CAD build for the part. Positions are in the model's coordinates, mm. A direction names the side the tool comes from. Coordinates: 2 decimals unless noted, no trailing zeros. Order: outer loops, then holes, each group sorted by start corner. A loop starts at its lowest first (then second) coordinate and runs counter-clockwise, first axis right, second up. Notation, with made-up numbers: M -13,-11.5 L -6,-11.5 A12 cw -6,1.5 Z; hole C -36,2 d10. An arc over 180 degrees is marked long. Write item = value, one per line.
from build123d import *

# Parameters (mm, degrees)
BOSS_EXTRUDE1_DEPTH = 20
SKETCH2_R           = 4
CUT_EXTRUDE1_DEPTH  = 15
LPATTERN1_COUNT     = 2
LPATTERN1_PITCH     = 170


with BuildPart() as part:
    # Sketch1 → Boss-Extrude1 (new body)
    with BuildSketch(Plane.XY):
        Polygon((0, 0), (184, 0), (184, 10), (0, 32.592359206), align=None)
    extrude(amount=BOSS_EXTRUDE1_DEPTH)

    # Sketch2 → Cut-Extrude1 (cut)
    with BuildSketch(Plane(origin=(3.942402661, 32.108293027, 0), x_dir=(0.9925461516413229, -0.12186934340514068, 0), z_dir=(0.12186934340514069, 0.992546151641323, 0))):
        with Locations(Location((173.909798468, -10, 0), (0, 0, 180))):
            Circle(SKETCH2_R)
    cut_extrude1 = extrude(amount=-CUT_EXTRUDE1_DEPTH, mode=Mode.SUBTRACT)

    # LPattern1: Cut-Extrude1 ×2
    with Locations(*[Vector(-0.9925461516413229, 0.12186934340514068, 0) * (i * LPATTERN1_PITCH) for i in range(1, LPATTERN1_COUNT)]):
        add(cut_extrude1, mode=Mode.SUBTRACT)


solid = part.part
(1) Slice it at B-B, the plane x = 158.5. Write the cut outline in (y, z).
Evaluation:
outline = M 0,0 L 13.13,0 L 13.13,20 L 0,20 Z
(2) Tool access for faces 4 (the face through (6.051, 16.737, 10.056)), 5 (the face through (70, 13, 20)): list every direction of +Z, -Z, +X, -X, +Y, -Y with a clear straight run to the whole face (end or side of a thin tool).
Evaluation:
face_4 = none
face_5 = +Z, +X, -X, +Y, -Y
(3) Slice it at A-A, the plane z = 3.75. Write the cut outline in (x, y).
Evaluation:
outline = M 0,0 L 184,0 L 184,10 L 0,32.59 Z
(4) Pull direction X, two halves, no side cores. Call faces 1 (the face through (3.135, 24.757, 11.201)), 2 (the face through (70, 13, 0)), 3 (the face through (184, 5, 10)): +X half, -X half, draft (parallel to the pull), parting line (faces both ways), or undercut.
Evaluation:
face_1 = undercut
face_2 = draft
face_3 = +X half
(5) Wall check: line 1 (X direction, y = 6.5, z = 7.5); line 2 (Y direction, x = 167, z = 16); line 3 (Y direction, x = 22, z = 16.25). Give the ranges that are in metal, low to high. Write a range as from..to.
Evaluation:
line_1 = 0..172.87, 179.16..184
line_2 = 0..12.09
line_3 = 0..29.89
(6) Pin check, flat tip, straight feed: pin 1 Ø12 at (x, z) = (145.5, 3.5) entering from +Y. Stop position of the tip, or through.
Evaluation:
pin_1 = 15.46
